Part model, mm, in its own coordinate system. Give positions to 0.01 mm unless a question says otherwise; leave off trailing zeros. Write each loop counter-clockwise with the first axis right and the second up, starting at its lowest first coordinate (ties: lowest second). Pieces come first, ordered by that corner, then holes. Notation, with made-up numbers: M -32.75,-4.5 L -4.75,-4.5 A27 cw -4.75,31.5 Z; hole C -14,8.25 d2. An arc over 180 degrees is marked long. Use a Markdown table: item, result.
```python
from build123d import *

# Parameters (mm, degrees)
SKETCH_1_W          = 100
SKETCH_1_H          = 100
EXTRUDE_1_DEPTH     = 14
HOLE_WIZARD_M12_1_D = 10.2
FILLET_1_R          = 10


with BuildPart() as part:
    # 草图1 → 凸台-拉伸1 (new body)
    with BuildSketch(Plane.XY):
        Rectangle(SKETCH_1_W, SKETCH_1_H)
    extrude(amount=EXTRUDE_1_DEPTH)

    # M12 螺纹孔1 (through all)
    with Locations(Plane(origin=(13.416407865, -26.83281573, 14), x_dir=(1, 0, 0), z_dir=(0, 0, 1))):
        with Locations((0, 0), (-26.83281573, 53.66563146)):
            Hole(HOLE_WIZARD_M12_1_D / 2)

    # 圆角1
    fillet_1_edges = [part.edges().sort_by_distance(p)[0] for p in [
        (-50, 50, 7),
        (-50, -50, 7),
        (50, -50, 7),
        (50, 50, 7),
    ]]
    fillet(fillet_1_edges, radius=FILLET_1_R)


solid = part.part
```
1. Cut at B-B, the plane x = 17. Give the cut face in (y, z), then the cut area to 3 significant figures.
Findings below:
| item | result |
|---|---|
| outline | M -50,0 L -30.46,0 L -30.46,14 L -50,14 Z; M -23.2,0 L 50,0 L 50,14 L -23.2,14 Z |
| area | 1,300 mm2 |
2. Two-plate mould, pull along X, no slides. Class faces 1 (the flat face through (50, -1, 7)), 2 (the flat face through (-1, 1, 0)), 3 (the cylindrical face through (11.063, -31.357, 6.902)): released by +X, released by -X, zero draft, split by the parting line, or undercut.
Findings below:
| item | result |
|---|---|
| face 1 | released by +X |
| face 2 | zero draft |
| face 3 | undercut |
3. Drill centre lines: L1, parallel to Y at x = -11.5, z = 2.5; L2, parallel to X at y = 30, z = 7; L3, parallel to X at y = 25, z = 11. Where is each one in solid material? Low to high.
Findings below:
| item | result |
|---|---|
| L1 | -50 to 22.11, 31.56 to 50 |
| L2 | -50 to -17.41, -9.42 to 50 |
| L3 | -50 to -18.18, -8.66 to 50 |
4. Cut at C-C, the plane z = 11.5. Give the cut face in (x, y).
Findings below:
| item | result |
|---|---|
| outline | M -50,-40 A10 ccw -40,-50 L 40,-50 A10 ccw 50,-40 L 50,40 A10 ccw 40,50 L -40,50 A10 ccw -50,40 Z; hole C -13.42,26.83 d10.2; hole C 13.42,-26.83 d10.2 |
5. Cut at A-A, the plane y = -29.5. Give the cut face in (x, z), then the cut area to 3 significant figures.
Findings below:
| item | result |
|---|---|
| outline | M -50,0 L 9.07,0 L 9.07,14 L -50,14 Z; M 17.76,0 L 50,0 L 50,14 L 17.76,14 Z |
| area | 1,280 mm2 |
